Source: CAD feature listing. Evaluate the final solid. Frame: model axes, mm. A direction names the side the tool comes from. Give positions to 0.01 mm unless a question says otherwise; leave off trailing zeros. Order: outer loops, then holes, each group sorted by start corner. A loop starts at its lowest first (then second) coordinate and runs counter-clockwise, first axis right, second up. Notation, with made-up numbers: M 43,89 L 55,89 A32 ccw 55,126 Z; hole C 3,-15.5 d1. An arc over 180 degrees is marked long. Use CSV: the item, a comma, the result in double quotes. Start each with the question number.
1. Mould query, pull axis Y, two halves, no side actions, for faces 1 (the flat face through (-10, 0, 172)), 2 (the cylindrical face through (12.47, 1.38, 177.35)), 3 (the cylindrical face through (12.465, -5.885, 185.434)). Classes: released by +Y, released by -Y, zero draft, split by the parting line, or undercut.
2. Reachability of faces 4 (the flat face through (0, 0, 156)), 5 (the flat face through (-5, 0, 15)), 6 (the cylindrical face through (-7.493, 0.33, 76.231)), 7 (the flat face through (5, 0, 15)), 8 (the flat face through (-4, -8, 155)) from +Z, -Z, +X, -X, +Y, -Y: full face, straight path, thin tool, end or side. Return the list, or none.
3. Section query A-A, the plane x = 0. Return the cut outline in (y, z).
4. Section query B-B, the plane z = 60.5. Return the cut outline in (x, y), plus the area to 3 significant figures.
5. Line query: line 1 along Z through (x, y) = (12.7, 0); line 2 along Z through (x, y) = (0.5, 0); line 3 along Z through (x, y) = (3.5, 3.5). Output: solid intervals per line, ascending. Write a range as [from, to].
6. Pin query (flat end, axial travel): P1, Ø1.5, axis at x = -1.5, z = 29, coming from the +Y side; P2, Ø8, axis at x = 4, y = 1.5, coming from the +Z side; P3, Ø3, axis at x = 5, y = 0.5, coming from the -Z side; P4, Ø5, axis at x = -3.5, y = -1, coming from the -Z side. Return the tip coordinate at first contact, or that it passes through.
from build123d import *

# Parameters (mm, degrees)
SKETCH1_R               = 7.5
BOSS_EXTRUDE1_DEPTH     = 150
SKETCH2_W               = 30
SKETCH2_H               = 16
BOSS_EXTRUDE2_DEPTH     = 38
SKETCH3_W               = 20
SKETCH3_H               = 19.358131828
CUT_EXTRUDE1_DEPTH      = 32
CUT_EXTRUDE2_DEPTH      = 191.546582231
CUT_EXTRUDE2_DEPTH_BACK = 191.546582231
SKETCH4_R               = 3
CUT_EXTRUDE3_DEPTH      = 189.76705221
CUT_EXTRUDE3_DEPTH_BACK = 189.76705221
SKETCH5_W               = 4.5
SKETCH5_H               = 15
SKETCH5_W_2             = 19.942706309
CUT_EXTRUDE4_DEPTH      = 190.029098289
CUT_EXTRUDE4_DEPTH_BACK = 190.029098289
SKETCH6_R               = 3


with BuildPart() as part:
    # Sketch1 → Boss-Extrude1 (new body)
    with BuildSketch(Plane.XY):
        Circle(SKETCH1_R)
    extrude(amount=BOSS_EXTRUDE1_DEPTH)

    # Sketch2 → Boss-Extrude2 (add)
    with BuildSketch(Plane.XY.offset(150)):
        Rectangle(SKETCH2_W, SKETCH2_H)
    extrude(amount=BOSS_EXTRUDE2_DEPTH)

    # Sketch3 → Cut-Extrude1 (cut)
    with BuildSketch(Plane.XY.offset(188)):
        Rectangle(SKETCH3_W, SKETCH3_H)
    extrude(amount=-CUT_EXTRUDE1_DEPTH, mode=Mode.SUBTRACT)

    # Sketch4 → Cut-Extrude2 (cut, two sides: drawn at the far end of the back side and taken through both)
    with BuildSketch(Plane(origin=(15, 0, 0), x_dir=(0, 0, -1), z_dir=(1, 0, 0)).offset(-CUT_EXTRUDE2_DEPTH_BACK)):
        with Locations(Location((-180.014983451, 0, 0), (0, 0, 90))):
            Circle(SKETCH4_R)
        with BuildLine():
            Line((-180.014983451, 8), (-180.014983451, 17.706818894))
            Line((-180.014983451, 17.706818894), (-220.326825599, 17.706818894))
            Line((-220.326825599, 17.706818894), (-218.614105417, -20.299257523))
            Line((-218.614105417, -20.299257523), (-180.014983451, -8))
            ThreePointArc((-180.014983451, -8), (-188.014983451, 0), (-180.014983451, 8))
        make_face()
    extrude(amount=CUT_EXTRUDE2_DEPTH + CUT_EXTRUDE2_DEPTH_BACK, mode=Mode.SUBTRACT)

    # Sketch5 → Cut-Extrude3 (cut, two sides: drawn at the far end of the back side and taken through both)
    with BuildSketch(Plane(origin=(0, 0, 0), x_dir=(1, 0, 0), z_dir=(0, 1, 0)).offset(-CUT_EXTRUDE3_DEPTH_BACK)):
        with Locations((-5.25, -7.5)):
            Rectangle(SKETCH5_W, SKETCH5_H)
        with Locations((12.971353155, -7.5)):
            Rectangle(SKETCH5_W_2, SKETCH5_H)
    extrude(amount=CUT_EXTRUDE3_DEPTH + CUT_EXTRUDE3_DEPTH_BACK, mode=Mode.SUBTRACT)

    # Sketch6 → Cut-Extrude4 (cut, two sides: drawn at the far end of the back side and taken through both)
    with BuildSketch(Plane.ZY.offset(3).offset(-CUT_EXTRUDE4_DEPTH_BACK)):
        with Locations((7.5, 0)):
            Circle(SKETCH6_R)
        with BuildLine():
            Line((7.5, 7.5), (-1.727121044, 19.130973882))
            Line((-1.727121044, 19.130973882), (-13.960832092, -5.232772696))
            Line((-13.960832092, -5.232772696), (1.279468959, -23.272312715))
            Line((1.279468959, -23.272312715), (7.5, -7.5))
            ThreePointArc((7.5, -7.5), (0, 0), (7.5, 7.5))
        make_face()
    extrude(amount=CUT_EXTRUDE4_DEPTH + CUT_EXTRUDE4_DEPTH_BACK, mode=Mode.SUBTRACT)


solid = part.part
Result set:
1,face 1,"zero draft"
1,face 2,"undercut"
1,face 3,"released by -Y"
2,face 4,"+Z, +Y, -Y"
2,face 5,"-Z, -X, +Y, -Y"
2,face 6,"-Z"
2,face 7,"-Z, +X, +Y, -Y"
2,face 8,"+Z, -Z, +X, -X, -Y"
3,outline,"M -8,150 L -7.5,150 L -7.5,7.5 A7.5 ccw 7.5,7.5 L 7.5,150 L 8,150 L 8,156 L -8,156 Z; hole C 0,7.5 d6"
4,outline,"C 0,0 d15"
4,area,"177 mm2"
5,line 1,"[150, 177.01], [183.01, 188]"
5,line 2,"[0, 4.5], [10.5, 156]"
5,line 3,"[15, 156]"
6,P1,"y = 7.46"
6,P2,"z = 156"
6,P3,"z = 15"
6,P4,"z = 0"
